Here's how the part is built. I have some questions about the finished solid (model axes, mm). Face numbers are marked on the shaded views. Coordinates: 2 decimals unless noted, no trailing zeros. Write each loop counter-clockwise with the first axis right and the second up, starting at its lowest first coordinate (ties: lowest second). Pieces come first, ordered by that corner, then holes. Notation, with made-up numbers: (-34, 36.5) -> (-15, 36.5) arc R20 ccw to (-15, 40.5) -> close; hole circle Ø7 at (24.5, 15). An arc over 180 degrees is marked (long way). Use CSV: the item, a comma, the result in double quotes. Start each with the question number.
```python
from build123d import *

# Parameters (mm, degrees)
SKETCH1_W                  = 80
SKETCH1_H                  = 16
BOSS_EXTRUDE1_DEPTH        = 20
SKETCH2_R                  = 5
CUT_EXTRUDE1_DEPTH         = 20
SKETCH3_W                  = 12.438334811
SKETCH3_H                  = 2
CUT_EXTRUDE2_DEPTH         = 30
M6_TAPPED_HOLE1_AT_2_COUNT = 2
M6_TAPPED_HOLE1_AT_2_PITCH = 68
SKETCH7_R                  = 3.25
CUT_EXTRUDE3_DEPTH         = 30
SKETCH8_R                  = 5
CUT_EXTRUDE7_DEPTH         = 4


with BuildPart() as part:
    # Sketch1 → Boss-Extrude1 (new body)
    with BuildSketch(Plane.XY):
        with Locations((-40, 8)):
            Rectangle(SKETCH1_W, SKETCH1_H)
    extrude(amount=BOSS_EXTRUDE1_DEPTH)

    # Sketch2 → Cut-Extrude1 (cut)
    with BuildSketch(Plane.XZ):
        with Locations((-15, 10)):
            Circle(SKETCH2_R)
        with Locations((-65, 10)):
            Circle(SKETCH2_R)
    extrude(amount=-CUT_EXTRUDE1_DEPTH, mode=Mode.SUBTRACT)

    # Sketch3 → Cut-Extrude2 (cut)
    with BuildSketch(Plane.XZ):
        with Locations((-4.725841747, 10)):
            Rectangle(SKETCH3_W, SKETCH3_H)
        with Locations((-75.274158254, 10)):
            Rectangle(SKETCH3_W, SKETCH3_H)
    extrude(amount=-CUT_EXTRUDE2_DEPTH, mode=Mode.SUBTRACT)

    # Sketch4 → M6 Tapped Hole1 (revolve, cut)
    with BuildSketch(Plane(origin=(-6, 8, 9), x_dir=(0, -1, 0), z_dir=(1, 0, 0))):
        Polygon((0, 0), (0, 18.502151548), (2.5, 17), (2.5, 0), align=None)
    m6_tapped_hole1 = revolve(axis=Axis((-6, 8, 15.35), (0, 0, -1)), mode=Mode.SUBTRACT)

    # M6 Tapped Hole1 at 2: M6 Tapped Hole1 ×2
    with Locations(*[(-i * M6_TAPPED_HOLE1_AT_2_PITCH, 0, 0) for i in range(1, M6_TAPPED_HOLE1_AT_2_COUNT)]):
        add(m6_tapped_hole1, mode=Mode.SUBTRACT)

    # Sketch7 → Cut-Extrude3 (cut)
    with BuildSketch(Plane(origin=(0, 0, 11), x_dir=(-1, 0, 0), z_dir=(0, 0, -1))):
        with Locations((74, 8)):
            Circle(SKETCH7_R)
        with Locations((6, 8)):
            Circle(SKETCH7_R)
    extrude(amount=-CUT_EXTRUDE3_DEPTH, mode=Mode.SUBTRACT)

    # Sketch8 → Cut-Extrude7 (cut)
    with BuildSketch(Plane.XY.offset(20)):
        with Locations((-6, 8)):
            Circle(SKETCH8_R)
        with Locations((-74, 8)):
            Circle(SKETCH8_R)
    extrude(amount=-CUT_EXTRUDE7_DEPTH, mode=Mode.SUBTRACT)


solid = part.part
```
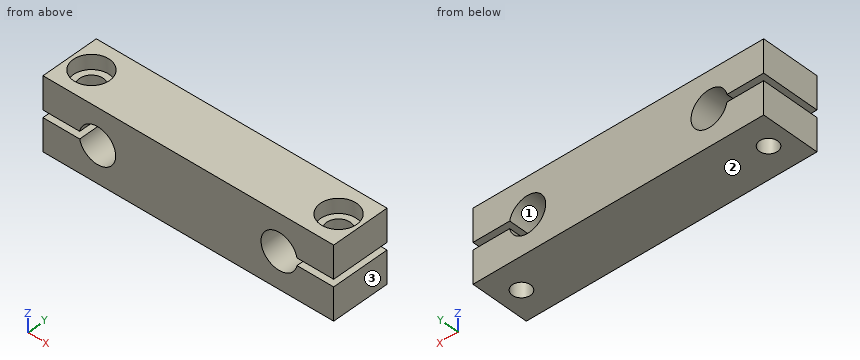
Item 1: I'm going to push a flat-ended pin straight in: pin 1 (3 mm diameter, centred on x = -73, y = 10, fed in from +Z). Where does the tip first touch, or does it pass through?
Item 2: I want a section at D-D on x = -16.5. Please give me the cut outline in (y, z).
Item 3: If I drill on line 1 along Y through (x, z) = (-74, 4); line 2 along Y through (x, z) = (-74, 18.05); line 3 along X through (y, z) = (10, 17.5), over which ranges is the centre line in solid material (lowest first)?
Item 4: I want a section at A-A on x = -68. Please give me the cut outline in (y, z).
Item 5: I want a section at C-C on y = 1.75. Please give me the cut outline in (x, z).
Item 6: I want a section at B-B on z = 12. Please give me the cut outline in (x, y).
Item 7: Thinking about a two-plate mould opening in Z: for the marked faces 1, 2 and 3, which applies, +Z half, -Z half, draft (parallel to the pull), parting line (faces both ways), or undercut?
Geometry says:
1,pin 1,"z = 16"
2,outline,"(0, 0) -> (16, 0) -> (16, 5.23) -> (0, 5.23) -> close; (0, 14.77) -> (16, 14.77) -> (16, 20) -> (0, 20) -> close"
3,line 1,"0 to 5.5, 10.5 to 16"
3,line 2,"0 to 3, 13 to 16"
3,line 3,"-80 to -78.58, -69.42 to -10.58, -1.42 to 0"
4,outline,"(0, 0) -> (16, 0) -> (16, 6) -> (0, 6) -> close; (0, 14) -> (16, 14) -> (16, 20) -> (0, 20) -> close"
5,outline,"(-80, 0) -> (0, 0) -> (0, 9) -> (-10.1, 9) arc R5 cw (long way) to (-10.1, 11) -> (0, 11) -> (0, 20) -> (-80, 20) -> (-80, 11) -> (-69.9, 11) arc R5 cw (long way) to (-69.9, 9) -> (-80, 9) -> close"
6,outline,"(-80, 0) -> (-69.58, 0) -> (-69.58, 16) -> (-80, 16) -> close; (-60.42, 0) -> (-19.58, 0) -> (-19.58, 16) -> (-60.42, 16) -> close; (-10.42, 0) -> (0, 0) -> (0, 16) -> (-10.42, 16) -> close; hole circle Ø6.5 at (-74, 8); hole circle Ø6.5 at (-6, 8)"
7,face 1,"undercut"
7,face 2,"-Z half"
7,face 3,"draft"
